from build123d import *

# Parameters (mm, degrees)
SKETCH1_R           = 85
BOSS_EXTRUDE1_DEPTH = 14
SKETCH2_R           = 55
BOSS_EXTRUDE2_DEPTH = 14
SKETCH3_R           = 49
CUT_EXTRUDE1_DEPTH  = 23
FILLET1_R           = 10
FILLET2_R           = 1
CHAMFER1_SIZE       = 1
SKETCH4_R           = 20
SKETCH4_R_2         = 6.75
CUT_EXTRUDE2_DEPTH  = 122.020659393
M12_TAPPED_HOLE1_D  = 10.2
CHAMFER2_SIZE       = 2


with BuildPart() as part:
    # Sketch1 → Boss-Extrude1 (new body)
    with BuildSketch(Plane(origin=(0, 0, 0), x_dir=(1, 0, 0), z_dir=(0, 1, 0))):
        with Locations(Location((0, 0, 0), (0, 0, 270))):
            Circle(SKETCH1_R)
    extrude(amount=BOSS_EXTRUDE1_DEPTH)

    # Sketch2 → Boss-Extrude2 (add)
    with BuildSketch(Plane(origin=(0, 14, 0), x_dir=(1, 0, 0), z_dir=(0, 1, 0))):
        with Locations(Location((0, 0, 0), (0, 0, 270))):
            Circle(SKETCH2_R)
    extrude(amount=BOSS_EXTRUDE2_DEPTH)

    # Sketch3 → Cut-Extrude1 (cut)
    with BuildSketch(Plane(origin=(0, 28, 0), x_dir=(1, 0, 0), z_dir=(0, 1, 0))):
        with Locations(Location((0, 0, 0), (0, 0, 270))):
            Circle(SKETCH3_R)
    extrude(amount=-CUT_EXTRUDE1_DEPTH, mode=Mode.SUBTRACT)

    # Fillet1
    fillet1_edges = [part.edges().sort_by_distance(p)[0] for p in [
        (0, 5, -49),
    ]]
    fillet(fillet1_edges, radius=FILLET1_R)

    # Fillet2
    fillet2_edges = [part.edges().sort_by_distance(p)[0] for p in [
        (0, 14, -55),
    ]]
    fillet(fillet2_edges, radius=FILLET2_R)

    # Chamfer1
    chamfer1_edges = [part.edges().sort_by_distance(p)[0] for p in [
        (0, 28, -55),
    ]]
    chamfer(chamfer1_edges, length=CHAMFER1_SIZE)

    # Sketch4 → Cut-Extrude2 (cut, through all)
    with BuildSketch(Plane(origin=(0, 14, 0), x_dir=(1, 0, 0), z_dir=(0, 1, 0))):
        with Locations((0, 90)):
            Circle(SKETCH4_R)
        with Locations(Location((-35, 60.621778265, 0), (0, 0, 270))):
            Circle(SKETCH4_R_2)
        with Locations(Location((35, 60.621778265, 0), (0, 0, 270))):
            Circle(SKETCH4_R_2)
        with Locations(Location((70, 0, 0), (0, 0, 270))):
            Circle(SKETCH4_R_2)
        with Locations(Location((35, -60.621778265, 0), (0, 0, 270))):
            Circle(SKETCH4_R_2)
        with Locations(Location((-35, -60.621778265, 0), (0, 0, 270))):
            Circle(SKETCH4_R_2)
        with Locations(Location((-70, 0, 0), (0, 0, 270))):
            Circle(SKETCH4_R_2)
    extrude(amount=-CUT_EXTRUDE2_DEPTH, mode=Mode.SUBTRACT)

    # M12 Tapped Hole1 (through all)
    with Locations(Plane(origin=(0, 14, 0), x_dir=(1, 0, 0), z_dir=(0, 1, 0))):
        with Locations((-60.621778265, -35), (60.621778265, 35)):
            Hole(M12_TAPPED_HOLE1_D / 2)

    # Chamfer2
    chamfer2_edges = [part.edges().sort_by_distance(p)[0] for p in [
        (0, 0, 85),
        (0, 0, -70),
    ]]
    chamfer(chamfer2_edges, length=CHAMFER2_SIZE)


solid = part.part
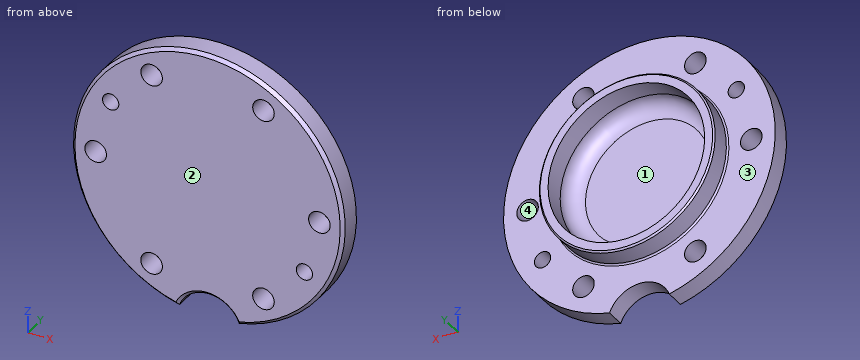
The model under review builds one solid part; all positions refer to its coordinate system, in mm. Face numbers are marked on the shaded views. A direction names the side the tool comes from. Round coordinates to 2 decimals unless told otherwise and drop trailing zeros. Loops run counter-clockwise (first coordinate to the right, second up) from the corner with the lowest first, then second, coordinate; pieces in that order, holes last. Notation, with made-up numbers: (-16, -10) -> (9, -10) arc R16 cw to (9, 14) -> close; hole circle Ø3 at (-20.5, 37). An arc over 180 degrees is marked (long way). Return JSON: item names as keys, results as strings.
(1) Add section A-A on z = 0. Write out the cut boundary in (x, y), plus the area to 3 significant figures.
Solved:
{"outline": "(-85, 2) -> (-83, 0) -> (-76.75, 0) -> (-76.75, 14) -> (-85, 14) -> close; (-63.25, 0) -> (63.25, 0) -> (63.25, 14) -> (56, 14) arc R1 cw to (55, 15) -> (55, 27) -> (54, 28) -> (49, 28) -> (49, 15) arc R10 cw to (39, 5) -> (-39, 5) arc R10 cw to (-49, 15) -> (-49, 28) -> (-54, 28) -> (-55, 27) -> (-55, 15) arc R1 cw to (-56, 14) -> (-63.25, 14) -> close; (76.75, 0) -> (83, 0) -> (85, 2) -> (85, 14) -> (76.75, 14) -> close", "area": "1,330 mm2"}
(2) The part is to be moulded in two halves that separate along X. For the marked faces 1 and 2, say which applies: released by +X, released by -X, zero draft, split by the parting line, or undercut.
Solved:
{"face 1": "undercut", "face 2": "zero draft"}
(3) Add section B-B on x = 0. Write out the cut boundary in (y, z).
Solved:
{"outline": "(0, -68) -> (2, -70) -> (14, -70) -> (14, -56) arc R1 cw to (15, -55) -> (27, -55) -> (28, -54) -> (28, -49) -> (15, -49) arc R10 cw to (5, -39) -> (5, 39) arc R10 cw to (15, 49) -> (28, 49) -> (28, 54) -> (27, 55) -> (15, 55) arc R1 cw to (14, 56) -> (14, 85) -> (2, 85) -> (0, 83) -> close"}
(4) For the marked faces 3 and 4, list the 3-axis set-ups (+Z, -Z, +X, -X, +Y, -Y) from which the entire face can be reached by the end or side of a thin tool; tool diameter is ignored.
Solved:
{"face 3": "+Y", "face 4": "+Y, -Y"}
(5) Add section C-C on y = 23. Write out the cut boundary in (x, z), plus the area to 3 significant figures.
Solved:
{"outline": "circle Ø110 at (0, 0); hole circle Ø98 at (0, 0)", "area": "1,960 mm2"}
(6) For pin 1 (1.5 mm diameter, centred on x = -18, y = 13.5, fed in from +Z); pin 2 (8 mm diameter, centred on y = 12, z = 49.5, fed in from -X); pin 3 (16.5 mm diameter, centred on x = -60.62, z = 35, fed in from +Y), all flat-tipped, find the tip position at first contact; note any pin that passes through.
Solved:
{"pin 1": "z = 83.23", "pin 2": "x = -71.8", "pin 3": "y = 14"}
(7) For line 1 (X direction, y = 4, z = -64); line 2 (X direction, y = 11, z = 35); line 3 (X direction, y = 9.75, z = -2.5), list the stretches that pass through material, from the lowest coordinate up.
Solved:
{"line 1": "-55.94 to -40.84, -29.16 to 29.16, 40.84 to 55.94", "line 2": "-77.46 to -65.72, -55.52 to -33.09, 33.09 to 77.46", "line 3": "-84.96 to -76.27, -63.73 to -47.45, 47.45 to 63.73, 76.27 to 84.96"}
(8) Add section D-D on x = -31.5. State how many separate pieces and enclosed holes the cut face has, plus the area to 3 significant figures.
Solved:
{"separate pieces": "3", "enclosed holes": "0", "area": "1,480 mm2"}
